from build123d import *

# Parameters (mm, degrees)
SKETCH1_W           = 230
SKETCH1_H           = 30
SKETCH1_R           = 3.25
BOSS_EXTRUDE1_DEPTH = 4
CHAMFER1_SIZE       = 2


with BuildPart() as part:
    # Sketch1 → Boss-Extrude1 (new body)
    with BuildSketch(Plane.XY):
        Rectangle(SKETCH1_W, SKETCH1_H)
        with Locations((-105, 0)):
            Circle(SKETCH1_R, mode=Mode.SUBTRACT)
        with Locations((-75, 0)):
            Circle(SKETCH1_R, mode=Mode.SUBTRACT)
        with Locations((20, 0)):
            Circle(SKETCH1_R, mode=Mode.SUBTRACT)
        with Locations((95, 0)):
            Circle(SKETCH1_R, mode=Mode.SUBTRACT)
    extrude(amount=BOSS_EXTRUDE1_DEPTH)

    # Chamfer1
    chamfer1_edges = [part.edges().sort_by_distance(p)[0] for p in [
        (-115, 15, 2),
        (115, 15, 2),
        (115, -15, 2),
        (-115, -15, 2),
    ]]
    chamfer(chamfer1_edges, length=CHAMFER1_SIZE)


solid = part.part
CAD build for the part. Positions are in the model's coordinates, mm. Round coordinates to 2 decimals unless told otherwise and drop trailing zeros. Loops run counter-clockwise (first coordinate to the right, second up) from the corner with the lowest first, then second, coordinate; pieces in that order, holes last.
(1) Cut at B-B (x = 95). Give the cut face in (y, z).
(2) Two-plate mould, pull along X, no slides. Class faces 1 (the flat face through (115, 0, 2)), 2 (the flat face through (-2, 0, 0)), 3 (the cylindrical face through (16.753, 0.143, 1.972)): +X half, -X half, draft (parallel to the pull), parting line (faces both ways), or undercut.
(3) Cut at A-A (z = 0.75). Give the cut face in (x, y), plus the area to 3 significant figures.
(4) Wall check: line 1 along Y through (x, z) = (95, 1.1); line 2 along X through (y, z) = (-1, 3.65); line 3 along X through (y, z) = (-1.5, 2.9). Give the ranges that are in metal, low to high.
(5) Cut at C-C (y = 0). Give the cut face in (x, z), plus the area to 3 significant figures.
Findings below:
1. outline: (-15, 0) - (-3.25, 0) - (-3.25, 4) - (-15, 4) - close; (3.25, 0) - (15, 0) - (15, 4) - (3.25, 4) - close
2. face 1: +X half
2. face 2: draft
2. face 3: undercut
3. outline: (-115, -13) - (-113, -15) - (113, -15) - (115, -13) - (115, 13) - (113, 15) - (-113, 15) - (-115, 13) - close; hole circle Ø6.5 at (-105, 0); hole circle Ø6.5 at (-75, 0); hole circle Ø6.5 at (20, 0); hole circle Ø6.5 at (95, 0)
3. area: 6,760 mm2
4. line 1: y = -15 to -3.25, 3.25 to 15
4. line 2: x = -115 to -108.09, -101.91 to -78.09, -71.91 to 16.91, 23.09 to 91.91, 98.09 to 115
4. line 3: x = -115 to -107.88, -102.12 to -77.88, -72.12 to 17.12, 22.88 to 92.12, 97.88 to 115
5. outline: (-115, 0) - (-108.25, 0) - (-108.25, 4) - (-115, 4) - close; (-101.75, 0) - (-78.25, 0) - (-78.25, 4) - (-101.75, 4) - close; (-71.75, 0) - (16.75, 0) - (16.75, 4) - (-71.75, 4) - close; (23.25, 0) - (91.75, 0) - (91.75, 4) - (23.25, 4) - close; (98.25, 0) - (115, 0) - (115, 4) - (98.25, 4) - close
5. area: 816 mm2
